Here's how the part is built. I have some questions about the finished solid (model axes, mm). Face numbers are marked on the shaded views. Give positions to 0.01 mm unless a question says otherwise; leave off trailing zeros. Loops run counter-clockwise (first coordinate to the right, second up) from the corner with the lowest first, then second, coordinate; pieces in that order, holes last. Notation, with made-up numbers: (-38, -16) -> (-25, -16) arc R12 cw to (-25, 3) -> close; hole circle Ø7 at (19, -29). An arc over 180 degrees is marked (long way). Answer in a Markdown table with one row per item. Add a question column.
Item 1: If I drill on line 1 (X direction, y = 0.5, z = -6); line 2 (X direction, y = 0.95, z = -7); line 3 (Z direction, x = -1.75, y = 0.55), over which ranges is the centre line in solid material (lowest first)?
Item 2: If we section it at C-C (x = -2.5): Write out the boundary of the cut face in (y, z).
Item 3: If we section it at B-B (y = 0.85): Write out the boundary of the cut face in (x, z), then the cut area to 3 significant figures.
Item 4: If we section it at A-A (z = -6): Write out the boundary of the cut face in (x, y).
Item 5: We'd pull the mould along Z, two halves only. Please class the marked faces 1, 2 and 3: released by +Z, released by -Z, zero draft, split by the parting line, or undercut.
```python
from build123d import *

# Parameters (mm, degrees)
SKETCH1_W                      = 10
SKETCH1_H                      = 20
BOSS_EXTRUDE1_DEPTH            = 1.5
CHAMFER1_SIZE                  = 1
F_2_5_2_5_DIAMETER_HOLE1_D     = 2.5
F_2_5_2_5_DIAMETER_HOLE1_DEPTH = 10
F_2_5_2_5_DIAMETER_HOLE1_TIP   = 0.751075774


with BuildPart() as part:
    # Sketch1 → Boss-Extrude1 (new body)
    with BuildSketch(Plane(origin=(0, 0, 0), x_dir=(1, 0, 0), z_dir=(0, 1, 0))):
        Rectangle(SKETCH1_W, SKETCH1_H)
    extrude(amount=BOSS_EXTRUDE1_DEPTH)

    # Chamfer1
    chamfer1_edges = [part.edges().sort_by_distance(p)[0] for p in [
        (5, 0.75, 10),
        (-5, 0.75, 10),
        (-5, 0.75, -10),
        (5, 0.75, -10),
    ]]
    chamfer(chamfer1_edges, length=CHAMFER1_SIZE)

    # Ø2.5 (2.5) Diameter Hole1
    with Locations(Plane(origin=(-2.5, 1.5, -6), x_dir=(0, 0, 1), z_dir=(0, 1, 0))):
        with Locations((0, 0), (0, 5)):
            Hole(F_2_5_2_5_DIAMETER_HOLE1_D / 2, depth=F_2_5_2_5_DIAMETER_HOLE1_DEPTH)
            with Locations((0, 0, -(F_2_5_2_5_DIAMETER_HOLE1_DEPTH + F_2_5_2_5_DIAMETER_HOLE1_TIP / 2))):  # 118° drill point
                Cone(0, F_2_5_2_5_DIAMETER_HOLE1_D / 2, F_2_5_2_5_DIAMETER_HOLE1_TIP, mode=Mode.SUBTRACT)


solid = part.part
```
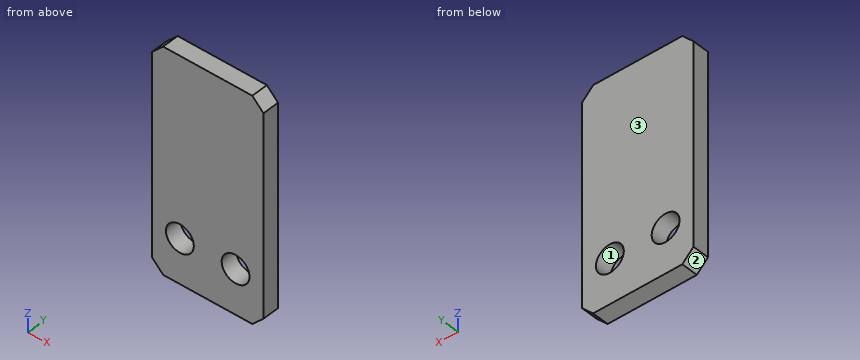
Recorded:
| question | item | result |
|---|---|---|
| 1 | line 1 | x = -5 to -3.75, -1.25 to 1.25, 3.75 to 5 |
| 1 | line 2 | x = -5 to -3.25, -1.75 to 1.75, 3.25 to 5 |
| 1 | line 3 | z = -10 to -7, -5 to 10 |
| 2 | outline | (0, -10) -> (1.5, -10) -> (1.5, -7.25) -> (0, -7.25) -> close; (0, -4.75) -> (1.5, -4.75) -> (1.5, 10) -> (0, 10) -> close |
| 3 | outline | (-5, -9) -> (-4, -10) -> (4, -10) -> (5, -9) -> (5, 9) -> (4, 10) -> (-4, 10) -> (-5, 9) -> close; hole circle Ø2.5 at (-2.5, -6); hole circle Ø2.5 at (2.5, -6) |
| 3 | area | 188 mm^2 |
| 4 | outline | (-5, 0) -> (-3.75, 0) -> (-3.75, 1.5) -> (-5, 1.5) -> close; (-1.25, 0) -> (1.25, 0) -> (1.25, 1.5) -> (-1.25, 1.5) -> close; (3.75, 0) -> (5, 0) -> (5, 1.5) -> (3.75, 1.5) -> close |
| 5 | face 1 | undercut |
| 5 | face 2 | released by -Z |
| 5 | face 3 | zero draft |
